from build123d import *

# Parameters (mm, degrees)
SKETCH1_W                       = 64.5
SKETCH1_H                       = 56
BOSS_EXTRUDE1_DEPTH             = 25
CUT_EXTRUDE1_REACH              = 51.488
SKETCH2_W                       = 62.5
SKETCH2_H                       = 52
CUT_EXTRUDE2_REACH              = 76.627
SKETCH3_R                       = 4
SKETCH3_R_2                     = 1.5
CUT_EXTRUDE3_REACH              = 71.29
SKETCH4_R                       = 4
SKETCH4_R_2                     = 1.5
FILLET3_R                       = 2
BOSS_EXTRUDE2_REACH             = 51.488
SKETCH5_W                       = 1.5
SKETCH5_H                       = 25
BOSS_EXTRUDE2_DIRECTION_2_REACH = 51.488
FILLET4_R                       = 2
SKETCH6_R                       = 1.5
SKETCH6_R_2                     = 4
CUT_EXTRUDE5_DEPTH              = 1.5


with BuildPart() as part:
    # Sketch1 → Boss-Extrude1 (new body)
    with BuildSketch(Plane.XY):
        Rectangle(SKETCH1_W, SKETCH1_H)
    extrude(amount=BOSS_EXTRUDE1_DEPTH)

    # Sketch2 → Cut-Extrude1 (cut, up to next)
    with BuildSketch(Plane.XY.offset(25), mode=Mode.PRIVATE) as cut_extrude1_sk1:
        with Locations((-1, 0)):
            Rectangle(SKETCH2_W, SKETCH2_H)
    cut_extrude1_tool1 = extrude(cut_extrude1_sk1.sketch, amount=-CUT_EXTRUDE1_REACH, mode=Mode.PRIVATE) & part.part
    add(cut_extrude1_tool1.solids().sort_by_distance((-1, 0, 25))[0], mode=Mode.SUBTRACT)

    # Sketch3 → Cut-Extrude2 (cut, up to next)
    with BuildSketch(Plane(origin=(32.25, 0, 0), x_dir=(0, 0, -1), z_dir=(1, 0, 0)), mode=Mode.PRIVATE) as cut_extrude2_sk1:
        with Locations((-12.5, 0)):
            Circle(SKETCH3_R)
    cut_extrude2_tool1 = extrude(cut_extrude2_sk1.sketch, amount=-CUT_EXTRUDE2_REACH, mode=Mode.PRIVATE) & part.part
    # Sketch3 → Cut-Extrude2 (cut, up to next)
    with BuildSketch(Plane(origin=(32.25, 0, 0), x_dir=(0, 0, -1), z_dir=(1, 0, 0)), mode=Mode.PRIVATE) as cut_extrude2_sk2:
        with Locations((-5.5, 0)):
            Circle(SKETCH3_R_2)
    cut_extrude2_tool2 = extrude(cut_extrude2_sk2.sketch, amount=-CUT_EXTRUDE2_REACH, mode=Mode.PRIVATE) & part.part
    # Sketch3 → Cut-Extrude2 (cut, up to next)
    with BuildSketch(Plane(origin=(32.25, 0, 0), x_dir=(0, 0, -1), z_dir=(1, 0, 0)), mode=Mode.PRIVATE) as cut_extrude2_sk3:
        with Locations((-12.5, 18.6)):
            Circle(SKETCH3_R_2)
    cut_extrude2_tool3 = extrude(cut_extrude2_sk3.sketch, amount=-CUT_EXTRUDE2_REACH, mode=Mode.PRIVATE) & part.part
    # Sketch3 → Cut-Extrude2 (cut, up to next)
    with BuildSketch(Plane(origin=(32.25, 0, 0), x_dir=(0, 0, -1), z_dir=(1, 0, 0)), mode=Mode.PRIVATE) as cut_extrude2_sk4:
        with Locations((-12.5, -7)):
            Circle(SKETCH3_R_2)
    cut_extrude2_tool4 = extrude(cut_extrude2_sk4.sketch, amount=-CUT_EXTRUDE2_REACH, mode=Mode.PRIVATE) & part.part
    # Sketch3 → Cut-Extrude2 (cut, up to next)
    with BuildSketch(Plane(origin=(32.25, 0, 0), x_dir=(0, 0, -1), z_dir=(1, 0, 0)), mode=Mode.PRIVATE) as cut_extrude2_sk5:
        with Locations((-19.5, 0)):
            Circle(SKETCH3_R_2)
    cut_extrude2_tool5 = extrude(cut_extrude2_sk5.sketch, amount=-CUT_EXTRUDE2_REACH, mode=Mode.PRIVATE) & part.part
    # Sketch3 → Cut-Extrude2 (cut, up to next)
    with BuildSketch(Plane(origin=(32.25, 0, 0), x_dir=(0, 0, -1), z_dir=(1, 0, 0)), mode=Mode.PRIVATE) as cut_extrude2_sk6:
        with Locations((-12.5, 7)):
            Circle(SKETCH3_R_2)
    cut_extrude2_tool6 = extrude(cut_extrude2_sk6.sketch, amount=-CUT_EXTRUDE2_REACH, mode=Mode.PRIVATE) & part.part
    # Sketch3 → Cut-Extrude2 (cut, up to next)
    with BuildSketch(Plane(origin=(32.25, 0, 0), x_dir=(0, 0, -1), z_dir=(1, 0, 0)), mode=Mode.PRIVATE) as cut_extrude2_sk7:
        with Locations(Location((-12.5, -18.6, 0), (0, 0, 90))):
            Circle(SKETCH3_R_2)
    cut_extrude2_tool7 = extrude(cut_extrude2_sk7.sketch, amount=-CUT_EXTRUDE2_REACH, mode=Mode.PRIVATE) & part.part
    add(cut_extrude2_tool1.solids().sort_by_distance((32.25, 0, 12.5))[0], mode=Mode.SUBTRACT)
    add(cut_extrude2_tool2.solids().sort_by_distance((32.25, 0, 5.5))[0], mode=Mode.SUBTRACT)
    add(cut_extrude2_tool3.solids().sort_by_distance((32.25, 18.6, 12.5))[0], mode=Mode.SUBTRACT)
    add(cut_extrude2_tool4.solids().sort_by_distance((32.25, -7, 12.5))[0], mode=Mode.SUBTRACT)
    add(cut_extrude2_tool5.solids().sort_by_distance((32.25, 0, 19.5))[0], mode=Mode.SUBTRACT)
    add(cut_extrude2_tool6.solids().sort_by_distance((32.25, 7, 12.5))[0], mode=Mode.SUBTRACT)
    add(cut_extrude2_tool7.solids().sort_by_distance((32.25, -18.6, 12.5))[0], mode=Mode.SUBTRACT)

    # Sketch4 → Cut-Extrude3 (cut, up to next)
    with BuildSketch(Plane.XZ.offset(28), mode=Mode.PRIVATE) as cut_extrude3_sk1:
        with Locations(Location((-19.75, 12.5, 0), (0, 0, 270))):
            Circle(SKETCH4_R)
    cut_extrude3_tool1 = extrude(cut_extrude3_sk1.sketch, amount=-CUT_EXTRUDE3_REACH, mode=Mode.PRIVATE) & part.part
    # Sketch4 → Cut-Extrude3 (cut, up to next)
    with BuildSketch(Plane.XZ.offset(28), mode=Mode.PRIVATE) as cut_extrude3_sk2:
        with Locations(Location((-12.75, 12.5, 0), (0, 0, 270))):
            Circle(SKETCH4_R_2)
    cut_extrude3_tool2 = extrude(cut_extrude3_sk2.sketch, amount=-CUT_EXTRUDE3_REACH, mode=Mode.PRIVATE) & part.part
    # Sketch4 → Cut-Extrude3 (cut, up to next)
    with BuildSketch(Plane.XZ.offset(28), mode=Mode.PRIVATE) as cut_extrude3_sk3:
        with Locations(Location((-1.15, 12.5, 0), (0, 0, 270))):
            Circle(SKETCH4_R_2)
    cut_extrude3_tool3 = extrude(cut_extrude3_sk3.sketch, amount=-CUT_EXTRUDE3_REACH, mode=Mode.PRIVATE) & part.part
    # Sketch4 → Cut-Extrude3 (cut, up to next)
    with BuildSketch(Plane.XZ.offset(28), mode=Mode.PRIVATE) as cut_extrude3_sk4:
        with Locations(Location((15.72, 12.5, 0), (0, 0, 270))):
            Circle(SKETCH4_R_2)
    cut_extrude3_tool4 = extrude(cut_extrude3_sk4.sketch, amount=-CUT_EXTRUDE3_REACH, mode=Mode.PRIVATE) & part.part
    # Sketch4 → Cut-Extrude3 (cut, up to next)
    with BuildSketch(Plane.XZ.offset(28), mode=Mode.PRIVATE) as cut_extrude3_sk5:
        with Locations(Location((-19.75, 5.5, 0), (0, 0, 270))):
            Circle(SKETCH4_R_2)
    cut_extrude3_tool5 = extrude(cut_extrude3_sk5.sketch, amount=-CUT_EXTRUDE3_REACH, mode=Mode.PRIVATE) & part.part
    # Sketch4 → Cut-Extrude3 (cut, up to next)
    with BuildSketch(Plane.XZ.offset(28), mode=Mode.PRIVATE) as cut_extrude3_sk6:
        with Locations(Location((-26.75, 12.5, 0), (0, 0, 270))):
            Circle(SKETCH4_R_2)
    cut_extrude3_tool6 = extrude(cut_extrude3_sk6.sketch, amount=-CUT_EXTRUDE3_REACH, mode=Mode.PRIVATE) & part.part
    # Sketch4 → Cut-Extrude3 (cut, up to next)
    with BuildSketch(Plane.XZ.offset(28), mode=Mode.PRIVATE) as cut_extrude3_sk7:
        with Locations(Location((-19.75, 19.5, 0), (0, 0, 270))):
            Circle(SKETCH4_R_2)
    cut_extrude3_tool7 = extrude(cut_extrude3_sk7.sketch, amount=-CUT_EXTRUDE3_REACH, mode=Mode.PRIVATE) & part.part
    cut_extrude3_1 = cut_extrude3_tool1.solids().sort_by_distance((-19.75, -28, 12.5))[0]
    add(cut_extrude3_1, mode=Mode.SUBTRACT)
    cut_extrude3_2 = cut_extrude3_tool2.solids().sort_by_distance((-12.75, -28, 12.5))[0]
    add(cut_extrude3_2, mode=Mode.SUBTRACT)
    cut_extrude3_3 = cut_extrude3_tool3.solids().sort_by_distance((-1.15, -28, 12.5))[0]
    add(cut_extrude3_3, mode=Mode.SUBTRACT)
    cut_extrude3_4 = cut_extrude3_tool4.solids().sort_by_distance((15.72, -28, 12.5))[0]
    add(cut_extrude3_4, mode=Mode.SUBTRACT)
    cut_extrude3_5 = cut_extrude3_tool5.solids().sort_by_distance((-19.75, -28, 5.5))[0]
    add(cut_extrude3_5, mode=Mode.SUBTRACT)
    cut_extrude3_6 = cut_extrude3_tool6.solids().sort_by_distance((-26.75, -28, 12.5))[0]
    add(cut_extrude3_6, mode=Mode.SUBTRACT)
    cut_extrude3_7 = cut_extrude3_tool7.solids().sort_by_distance((-19.75, -28, 19.5))[0]
    add(cut_extrude3_7, mode=Mode.SUBTRACT)
    cut_extrude3 = cut_extrude3_1 + cut_extrude3_2 + cut_extrude3_3 + cut_extrude3_4 + cut_extrude3_5 + cut_extrude3_6 + cut_extrude3_7  # Cut-Extrude3 as one shape, for the pattern or mirror that repeats it

    # Mirror1: Cut-Extrude3 across plane
    add(cut_extrude3.mirror(Plane.ZX), mode=Mode.SUBTRACT)

    # Fillet3
    fillet3_edges = [part.edges().sort_by_distance(p)[0] for p in [
        (32.25, -28, 12.5),
        (32.25, 28, 12.5),
    ]]
    fillet(fillet3_edges, radius=FILLET3_R)

    # Boss-Extrude2: up to this face of the body (flat: up to its plane)
    boss_extrude2_end = Plane(part.part.faces().sort_by_distance((-1, 28, 0.673145601))[0])
    # Sketch5 → Boss-Extrude2 (add, up to the picked face)
    with BuildSketch(Plane(origin=(0, 0, 0), x_dir=(1, 0, 0), z_dir=(0, 1, 0)), mode=Mode.PRIVATE) as boss_extrude2_sk1:
        with Locations((-33, -12.5)):
            Rectangle(SKETCH5_W, SKETCH5_H)
    boss_extrude2_tool1 = split(extrude(boss_extrude2_sk1.sketch, amount=BOSS_EXTRUDE2_REACH, mode=Mode.PRIVATE), bisect_by=boss_extrude2_end, keep=Keep.BOTH, mode=Mode.PRIVATE)
    add(boss_extrude2_tool1.solids().sort_by(Axis((-33, 0, 12.5), (0, 1, 0)))[0])

    # Boss-Extrude2 direction 2: up to this face of the body (flat: up to its plane)
    boss_extrude2_direction_2_end = Plane(part.part.faces().sort_by_distance((-1, -28, 0.673145601))[0])
    # Sketch5 → Boss-Extrude2 direction 2 (add, up to the picked face)
    with BuildSketch(Plane(origin=(0, 0, 0), x_dir=(1, 0, 0), z_dir=(0, 1, 0)), mode=Mode.PRIVATE) as boss_extrude2_direction_2_sk1:
        with Locations((-33, -12.5)):
            Rectangle(SKETCH5_W, SKETCH5_H)
    boss_extrude2_direction_2_tool1 = split(extrude(boss_extrude2_direction_2_sk1.sketch, amount=-BOSS_EXTRUDE2_DIRECTION_2_REACH, mode=Mode.PRIVATE), bisect_by=boss_extrude2_direction_2_end, keep=Keep.BOTH, mode=Mode.PRIVATE)
    add(boss_extrude2_direction_2_tool1.solids().sort_by(Axis((-33, 0, 12.5), (0, -1, 0)))[0])

    # Fillet4
    fillet4_edges = [part.edges().sort_by_distance(p)[0] for p in [
        (-33.75, 28, 12.5),
        (-33.75, -28, 12.5),
    ]]
    fillet(fillet4_edges, radius=FILLET4_R)

    # Sketch6 → Cut-Extrude5 (cut)
    with BuildSketch(Plane(origin=(-32.25, 0, 0), x_dir=(0, 0, -1), z_dir=(1, 0, 0))):
        with Locations((-12.5, -2.25)):
            Circle(SKETCH6_R)
        with Locations((-19.5, -9.25)):
            Circle(SKETCH6_R)
        with Locations((-5.5, -9.25)):
            Circle(SKETCH6_R)
        with Locations((-12.5, -16.25)):
            Circle(SKETCH6_R)
        with Locations((-12.5, -9.25)):
            Circle(SKETCH6_R_2)
    extrude(amount=-CUT_EXTRUDE5_DEPTH, mode=Mode.SUBTRACT)


solid = part.part
The model under review builds one solid part; all positions refer to its coordinate system, in mm. A direction names the side the tool comes from. Give positions to 0.01 mm unless a question says otherwise; leave off trailing zeros. Order: outer loops, then holes, each group sorted by start corner. A loop starts at its lowest first (then second) coordinate and runs counter-clockwise, first axis right, second up. Notation, with made-up numbers: M -16,82 L 4,82 A18 cw 4,99 Z; hole C 53.5,85 d11. An arc over 180 degrees is marked long. Answer in a Markdown table with one row per item. Add a question column.
1. Add section A-A on x = -1.15. State the section outline as (y, z) points, plus the area to 3 significant figures.
2. Add section D-D on y = 24. State the section outline as (x, z) points.
3. Mouldability with a two-part tool opening along X and no side actions: class faces 4 (the cylindrical face through (31.65, 27.43, 12.68)), 5 (the cylindrical face through (-33.18, 27.4, 12.32)), 6 (the cylindrical face through (17.207, -27.014, 12.695)), 7 (the cylindrical face through (-18.74, -27.01, 6.61)) as released by +X, released by -X, zero draft, split by the parting line, or undercut.
4. For pin 1 Ø3.5 at (x, z) = (-19.75, 5.5) entering from +Y, flat-tipped, find the tip position at first contact; note if it passes through.
5. Add section C-C on x = 22.5. State the section outline as (y, z) points.
6. Machinability: for faces 1 (the cylindrical face through (-32.99, -10.714, 5.825)), 2 (the flat face through (-32.25, 0, 13)), 3 (the cylindrical face through (31.3, -2.4, 15.7)), which of the approach directions +Z, -Z, +X, -X, +Y, -Y give a long, thin tool a straight path to every point of the face, cutting with its end or side? Answer none if there is none.
7. Add section B-B on z = 19.5. State the section outline as (x, y) points.
8. To check wall thickness, follow line 1 along X through (y, z) = (-24.5, 8.5); line 2 along Y through (x, z) = (5, 4.25); line 3 along Y through (x, z) = (-32.6, 12.5). State the ranges of each line that lie inside material, in increasing order.
The answers:
| question | item | result |
|---|---|---|
| 1 | outline | M -28,0 L -26,0 L -26,11 L -28,11 Z; M -28,14 L -26,14 L -26,25 L -28,25 Z; M 26,0 L 28,0 L 28,11 L 26,11 Z; M 26,14 L 28,14 L 28,25 L 26,25 Z |
| 1 | area | 88.0 mm2 |
| 2 | outline | M -33.75,0 L -32.25,0 L -32.25,25 L -33.75,25 Z; M 30.25,0 L 32.25,0 L 32.25,25 L 30.25,25 Z |
| 3 | face 4 | released by +X |
| 3 | face 5 | released by -X |
| 3 | face 6 | undercut |
| 3 | face 7 | undercut |
| 4 | pin 1 | y = 28 |
| 5 | outline | M -28,0 L -26,0 L -26,25 L -28,25 Z; M 26,0 L 28,0 L 28,25 L 26,25 Z |
| 6 | face 1 | -X |
| 6 | face 2 | +Z, -Z |
| 6 | face 3 | +X |
| 7 | outline | M -33.75,-26 A2 ccw -31.75,-28 L -21.25,-28 L -21.25,-26 L -32.25,-26 L -32.25,-10.75 L -33.75,-10.75 Z; M -33.75,-7.75 L -32.25,-7.75 L -32.25,26 L -21.25,26 L -21.25,28 L -31.75,28 A2 ccw -33.75,26 Z; M -18.25,-28 L 30.25,-28 A2 ccw 32.25,-26 L 32.25,-1.5 L 30.25,-1.5 L 30.25,-26 L -18.25,-26 Z; M -18.25,26 L 30.25,26 L 30.25,1.5 L 32.25,1.5 L 32.25,26 A2 ccw 30.25,28 L -18.25,28 Z |
| 8 | line 1 | -33.75 to -32.25, 30.25 to 32.25 |
| 8 | line 2 | -28 to -26, 26 to 28 |
| 8 | line 3 | -27.81 to -17.75, -14.75 to -13.25, -5.25 to -3.75, -0.75 to 27.81 |
